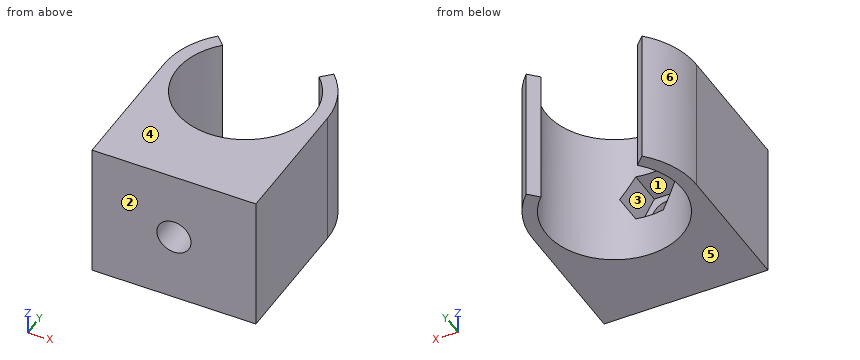
from build123d import *

# Parameters (mm, degrees)
EXTRUDE_1_DEPTH          = 20
HOLE_WIZARD_5_0_5_1_D    = 5
CUT_EXTRUDE_3_DEPTH      = 5
CUT_EXTRUDE_3_DEPTH_BACK = 5


with BuildPart() as part:
    # 草图1 → 凸台-拉伸1 (new body)
    with BuildSketch(Plane.XY):
        with BuildLine():
            Line((-12, 10), (-12, 20))
            ThreePointArc((-12, 20), (-11.08655439, 24.592201188), (-8.485281374, 28.485281374))
            Line((-8.485281374, 28.485281374), (-7.071067812, 27.071067812))
            ThreePointArc((-7.071067812, 27.071067812), (0, 10), (7.071067812, 27.071067812))
            Line((7.071067812, 27.071067812), (8.485281374, 28.485281374))
            ThreePointArc((8.485281374, 28.485281374), (11.08655439, 24.592201188), (12, 20))
            Line((12, 20), (12, 10))
            Line((12, 10), (12, 0))
            Line((12, 0), (-12, 0))
            Line((-12, 0), (-12, 10))
        make_face()
    extrude(amount=EXTRUDE_1_DEPTH)

    # Ø5.0 (5) 直径孔1 (through all)
    with Locations(Plane(origin=(0, 0, 0), x_dir=(-1, 0, 0), z_dir=(0, -1, 0))):
        with Locations((0, -10)):
            Hole(HOLE_WIZARD_5_0_5_1_D / 2)

    # 草图7 → 切除-拉伸3 (cut, two sides: drawn at the far end of the back side and taken through both)
    with BuildSketch(Plane(origin=(0, 10, 0), x_dir=(-1, 0, 0), z_dir=(0, -1, 0)).offset(-CUT_EXTRUDE_3_DEPTH_BACK)):
        Polygon((4.041451884, -10), (2.020725942, -6.5), (-2.020725942, -6.5), (-4.041451884, -10), (-2.020725942, -13.5), (2.020725942, -13.5), align=None)
    extrude(amount=CUT_EXTRUDE_3_DEPTH + CUT_EXTRUDE_3_DEPTH_BACK, mode=Mode.SUBTRACT)


solid = part.part
Geometry check sheet. Reference: the model listing, model coordinates, mm. Face numbers are marked on the shaded views. A direction names the side the tool comes from. Give positions to 0.01 mm unless a question says otherwise; leave off trailing zeros. Loops run counter-clockwise (first coordinate to the right, second up) from the corner with the lowest first, then second, coordinate; pieces in that order, holes last. Notation, with made-up numbers: (-3, 26) -> (16, 26) arc R26 cw to (16, 63) -> close; hole circle Ø8 at (77.5, -7.5). An arc over 180 degrees is marked (long way). Answer in a Markdown table with one row per item. Add a question column.
1) Set-up check for the marked faces 1 and 2: record each of +Z, -Z, +X, -X, +Y, -Y from which the full face is reachable in a straight line by a thin tool's end or side.
2) Material ranges on probe 1 along X at (y, z) = (20, 16); probe 2 along X at (y, z) = (2.75, 10); probe 3 along Z at (x, y) = (0, 2.15), recorded low to high. Write a range as from..to.
3) Cross-section at D-D on y = 22.25. Record the boundary of the cut face in (x, z).
4) Cross-section at B-B on y = 8.5. Record the boundary of the cut face in (x, z).
5) Gauge pin test, flat ends, axial feed: P1, Ø1.5, axis at x = -2.5, z = 3, coming from the +Y side; P2, Ø2, axis at y = 25.5, z = 10.5, coming from the +X side; P3, Ø5.5, axis at x = -1.5, z = 9.5, coming from the +Y side. Record the tip position at first contact, or that the pin passes through.
6) Draft check along Z on the marked faces 3, 4, 5 and 6. Enter one of: pulls with the +Z half, pulls with the -Z half, needs draft (parallel to the pull), parting line crosses it, or undercut.
7) Cross-section at A-A on x = 0. Record the boundary of the cut face in (y, z), and give its area (3 significant figures).
8) Cross-section at C-C on z = 18. Record the boundary of the cut face in (x, y), and give its area (3 significant figures).
Outcome:
| question | item | result |
|---|---|---|
| 1 | face 1 | +Y |
| 1 | face 2 | +Z, -Z, +X, -X, -Y |
| 2 | probe 1 | x = -12..-10, 10..12 |
| 2 | probe 2 | x = -12..-2.5, 2.5..12 |
| 2 | probe 3 | z = 0..7.5, 12.5..20 |
| 3 | outline | (-11.79, 0) -> (-9.74, 0) -> (-9.74, 20) -> (-11.79, 20) -> close; (9.74, 0) -> (11.79, 0) -> (11.79, 20) -> (9.74, 20) -> close |
| 4 | outline | (-12, 0) -> (12, 0) -> (12, 20) -> (-12, 20) -> close; hole (-4.04, 10) -> (-2.02, 6.5) -> (2.02, 6.5) -> (4.04, 10) -> (2.02, 13.5) -> (-2.02, 13.5) -> close |
| 5 | P1 | stops at y = 10.54 |
| 5 | P2 | stops at x = 11.12 |
| 5 | P3 | stops at y = 10.95 |
| 6 | face 3 | undercut |
| 6 | face 4 | pulls with the +Z half |
| 6 | face 5 | pulls with the -Z half |
| 6 | face 6 | needs draft |
| 7 | outline | (0, 0) -> (10, 0) -> (10, 6.5) -> (5, 6.5) -> (5, 7.5) -> (0, 7.5) -> close; (0, 12.5) -> (5, 12.5) -> (5, 13.5) -> (10, 13.5) -> (10, 20) -> (0, 20) -> close |
| 7 | area | 140 mm^2 |
| 8 | outline | (-12, 0) -> (12, 0) -> (12, 20) arc R12 ccw to (8.49, 28.49) -> (7.07, 27.07) arc R10 cw (long way) to (-7.07, 27.07) -> (-8.49, 28.49) arc R12 ccw to (-12, 20) -> close |
| 8 | area | 357 mm^2 |
